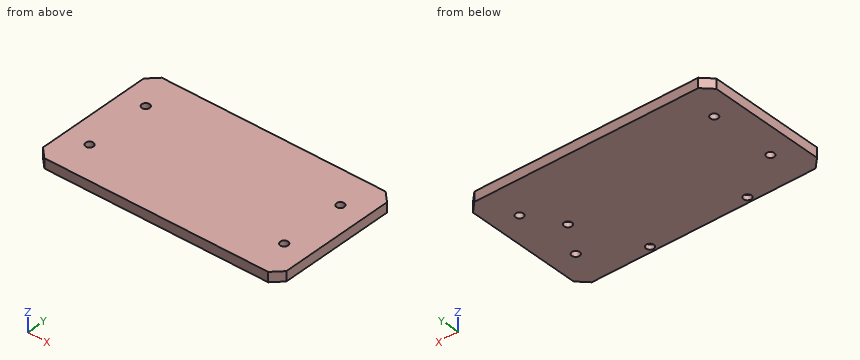
from build123d import *

# Parameters (mm, degrees)
BOSS_EXTRUDE1_DEPTH = 10
SKETCH6_R           = 4
CUT_EXTRUDE3_DEPTH  = 5
BOSS_EXTRUDE3_START = 5
SKETCH7_R           = 4
BOSS_EXTRUDE3_DEPTH = 5
SKETCH8_R           = 4
CUT_EXTRUDE4_DEPTH  = 5
SKETCH11_R          = 4
CUT_EXTRUDE5_DEPTH  = 10


with BuildPart() as part:
    # Sketch1 → Boss-Extrude1 (new body)
    with BuildSketch(Plane.XY):
        Polygon((-115, 70), (-125, 60), (-125, -60), (-115, -70), (115, -70), (125, -60), (125, 60), (115, 70), align=None)
    extrude(amount=BOSS_EXTRUDE1_DEPTH)

    # Sketch6 → Cut-Extrude3 (cut)
    with BuildSketch(Plane(origin=(0, 0, 0), x_dir=(-1, 0, 0), z_dir=(0, 0, -1))):
        with Locations((79.1, 0)):
            Circle(SKETCH6_R)
        with Locations(Location((-79.1, 0, 0), (0, 0, 180))):
            Circle(SKETCH6_R)
    extrude(amount=-CUT_EXTRUDE3_DEPTH, mode=Mode.SUBTRACT)

    # Sketch7 → Boss-Extrude3 (add)
    with BuildSketch(Plane(origin=(0, 0, 5), x_dir=(-1, 0, 0), z_dir=(0, 0, -1)).offset(BOSS_EXTRUDE3_START)):
        with Locations((79.1, 0)):
            Circle(SKETCH7_R)
    extrude(amount=-BOSS_EXTRUDE3_DEPTH)

    # Sketch8 → Cut-Extrude4 (cut)
    with BuildSketch(Plane(origin=(0, 0, 0), x_dir=(-1, 0, 0), z_dir=(0, 0, -1))):
        with Locations((-50, -64.1)):
            Circle(SKETCH8_R)
        with Locations(Location((50, -64.1, 0), (0, 0, 180))):
            Circle(SKETCH8_R)
    extrude(amount=-CUT_EXTRUDE4_DEPTH, mode=Mode.SUBTRACT)

    # Sketch11 → Cut-Extrude5 (cut)
    with BuildSketch(Plane.XY.offset(10)):
        with Locations((100, 33.5)):
            Circle(SKETCH11_R)
        with Locations(Location((-100, 33.5, 0), (0, 0, 180))):
            Circle(SKETCH11_R)
        with Locations((-100, -33.5)):
            Circle(SKETCH11_R)
        with Locations(Location((100, -33.5, 0), (0, 0, 180))):
            Circle(SKETCH11_R)
    extrude(amount=-CUT_EXTRUDE5_DEPTH, mode=Mode.SUBTRACT)


solid = part.part
Model file for the job. Use its own axes, mm. Give positions to 0.01 mm unless a question says otherwise; leave off trailing zeros. Order: outer loops, then holes, each group sorted by start corner. A loop starts at its lowest first (then second) coordinate and runs counter-clockwise, first axis right, second up. Notation, with made-up numbers: (86.25, -23) - (103.25, -23) arc R22 ccw to (103.25, 10) - close; hole circle Ø9 at (10, 87.5). An arc over 180 degrees is marked (long way). One line per item, written item: value.
Item 1: Slice it at A-A (x = 100). List the corners of the cut face in (y, z), then the cut area to 3 significant figures.
Response values:
outline: (-70, 0) - (-37.5, 0) - (-37.5, 10) - (-70, 10) - close; (-29.5, 0) - (29.5, 0) - (29.5, 10) - (-29.5, 10) - close; (37.5, 0) - (70, 0) - (70, 10) - (37.5, 10) - close
area: 1,240 mm2
Item 2: Wall check: line 1 (Y direction, x = -50, z = 4.5); line 2 (X direction, y = 37, z = 4.25). Give the ranges that are in metal, low to high.
Response values:
line 1: -70 to -68.1, -60.1 to 70
line 2: -125 to -101.94, -98.06 to 98.06, 101.94 to 125
Item 3: Slice it at B-B (y = 33.5). List the corners of the cut face in (x, z).
Response values:
outline: (-125, 0) - (-104, 0) - (-104, 10) - (-125, 10) - close; (-96, 0) - (96, 0) - (96, 10) - (-96, 10) - close; (104, 0) - (125, 0) - (125, 10) - (104, 10) - close
Item 4: Slice it at C-C (z = 3.25). List the corners of the cut face in (x, y).
Response values:
outline: (-125, -60) - (-115, -70) - (115, -70) - (125, -60) - (125, 60) - (115, 70) - (-115, 70) - (-125, 60) - close; hole circle Ø8 at (-100, -33.5); hole circle Ø8 at (-100, 33.5); hole circle Ø8 at (-50, -64.1); hole circle Ø8 at (50, -64.1); hole circle Ø8 at (79.1, 0); hole circle Ø8 at (100, -33.5); hole circle Ø8 at (100, 33.5)
Item 5: Slice it at D-D (y = -64.1). List the corners of the cut face in (x, z), then the cut area to 3 significant figures.
Response values:
outline: (-120.9, 0) - (-54, 0) - (-54, 5) - (-46, 5) - (-46, 0) - (46, 0) - (46, 5) - (54, 5) - (54, 0) - (120.9, 0) - (120.9, 10) - (-120.9, 10) - close
area: 2,340 mm2
